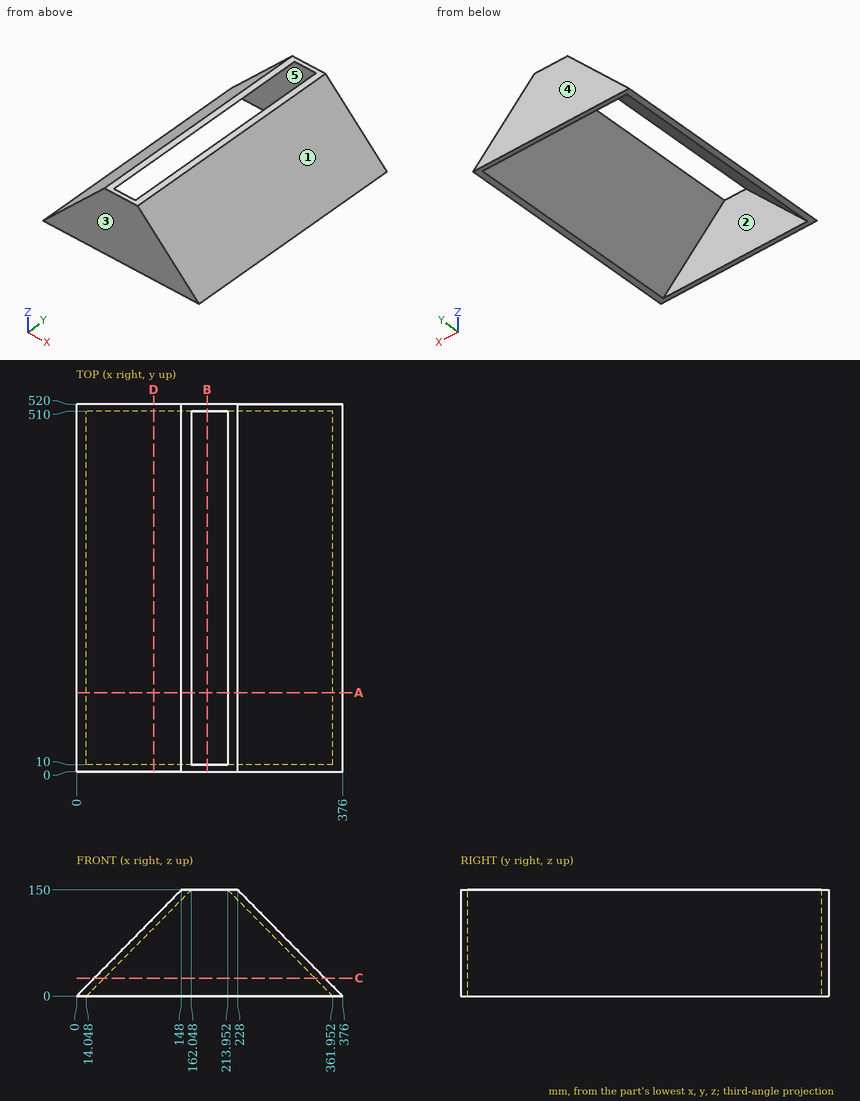
The figure shows three views and two pictorial views of one solid part (mm, origin at its lowest corner). Answer the questions. A direction names the side the tool comes from. Give positions to 0.01 mm unless a question says otherwise; leave off trailing zeros. Order: outer loops, then holes, each group sorted by start corner. A loop starts at its lowest first (then second) coordinate and runs counter-clockwise, first axis right, second up. Notation, with made-up numbers: (-35.5, -16.75) -> (3.5, -16.75) arc R13 ccw to (3.5, -10.75) -> close; hole circle Ø1 at (-27.75, -12). An arc over 180 degrees is marked (long way). One line per item, written item: value.
1) Find the intervals of material crossed by line 1 (Y direction, x = 232, z = 34.5); line 2 (X direction, y = 259, z = 139) (1 decimal); line 3 (X direction, y = 441, z = 88.5), in increasing order.
Reported:
line 1: y = 0 to 10, 510 to 520
line 2: x = 137.1 to 151.2, 224.8 to 238.9
line 3: x = 87.32 to 101.37, 274.63 to 288.68
2) Find section C-C, the plane z = 25.5. Determine the outline of the cut face in (x, y), plus the area to 3 significant figures.
Reported:
outline: (25.16, 0) -> (350.84, 0) -> (350.84, 520) -> (25.16, 520) -> close; hole (39.21, 10) -> (336.79, 10) -> (336.79, 510) -> (39.21, 510) -> close
area: 20,600 mm^2
3) A tool of negligible diameter and unlimited length cuts with its end or side. For the marked faces 1 and 2, from which of +Z, -Z, +X, -X, +Y, -Y can it reach the whole face along a straight path? Write none if from no direction.
Reported:
face 1: +Z, +X, +Y, -Y
face 2: -Z
4) Flat-ended cylindrical pins translate along their axes: P1, Ø10, axis at x = 52.5, y = 325, coming from the -Z side; P2, Ø2, axis at y = 394.5, z = 117, coming from the -X side; P3, Ø4, axis at y = 356.5, z = 22.5, coming from the -X side. Find the tip coordinate at first contact, or state that the pin passes through.
Reported:
P1: stops at z = 33.9
P2: stops at x = 114.45
P3: stops at x = 20.23
5) Find section D-D, the plane x = 109. Determine the outline of the cut face in (y, z) (3 decimals), plus the area to 3 significant figures.
Reported:
outline: (0, 0) -> (10, 0) -> (10, 96.235) -> (510, 96.235) -> (510, 0) -> (520, 0) -> (520, 110.473) -> (0, 110.473) -> close
area: 9,330 mm^2
6) Determine the mould class of the marked faces 3, 4 and 5 for opening direction Y: pulls with the +Y half, pulls with the -Y half, needs draft (parallel to the pull), parting line crosses it, or undercut.
Reported:
face 3: pulls with the -Y half
face 4: pulls with the +Y half
face 5: undercut
7) Find section B-B, the plane x = 184.5. Determine the outline of the cut face in (y, z).
Reported:
outline: (0, 0) -> (10, 0) -> (10, 150) -> (0, 150) -> close; (510, 0) -> (520, 0) -> (520, 150) -> (510, 150) -> close
8) Find section A-A, the plane y = 112. Determine the outline of the cut face in (x, z), plus the area to 3 significant figures.
Reported:
outline: (0, 0) -> (14.05, 0) -> (162.05, 150) -> (148, 150) -> close; (213.95, 150) -> (361.95, 0) -> (376, 0) -> (228, 150) -> close
area: 4,210 mm^2
